Design review of the part built by this model. Coordinates are the model's own, in mm. A direction names the side the tool comes from. Coordinates: 2 decimals unless noted, no trailing zeros. Order: outer loops, then holes, each group sorted by start corner. A loop starts at its lowest first (then second) coordinate and runs counter-clockwise, first axis right, second up. Notation, with made-up numbers: M 38,-27 L 85,-27 A17 ccw 85,0 Z; hole C 70,-38.5 d3. An arc over 180 degrees is marked long. Answer in a Markdown table with one row per item.
from build123d import *

# Parameters (mm, degrees)
SKETCH1_R           = 8.5
SKETCH1_R_2         = 1.5
BOSS_EXTRUDE1_DEPTH = 3
FILLET1_R           = 3


with BuildPart() as part:
    # Sketch1 → Boss-Extrude1 (new body)
    with BuildSketch(Plane(origin=(0, 0, 0), x_dir=(1, 0, 0), z_dir=(0, 1, 0))):
        Polygon((-11, 0), (11, 0), (20.489621783, 17.605313925), (20.489621783, 47.605313925), (8, 62), (-8, 62), (-20.509243816, 47.910305032), (-20.509243816, 17.610706132), align=None)
        with Locations(Location((7.519679741, 17.780252273, 0), (0, 0, 270))):
            Circle(SKETCH1_R, mode=Mode.SUBTRACT)
        with Locations(Location((6, 4, 0), (0, 0, 270))):
            Circle(SKETCH1_R_2, mode=Mode.SUBTRACT)
        with Locations(Location((-6, 4, 0), (0, 0, 90))):
            Circle(SKETCH1_R_2, mode=Mode.SUBTRACT)
        with Locations(Location((-5.25, 57.999859765, 0), (0, 0, 270))):
            Circle(SKETCH1_R_2, mode=Mode.SUBTRACT)
        with Locations(Location((5.25, 57.999859765, 0), (0, 0, 270))):
            Circle(SKETCH1_R_2, mode=Mode.SUBTRACT)
        with Locations(Location((-13.5, 37.605313925, 0), (0, 0, 270))):
            Circle(SKETCH1_R_2, mode=Mode.SUBTRACT)
        with Locations(Location((13.5, 37.605313925, 0), (0, 0, 270))):
            Circle(SKETCH1_R_2, mode=Mode.SUBTRACT)
        with BuildLine():
            Line((-8.730303993, 39.105313925), (8.730303993, 39.105313925))
            ThreePointArc((8.730303993, 39.105313925), (10.179901517, 41.34388933), (12.574074074, 42.518832133))
            ThreePointArc((12.574074074, 42.518832133), (0, 51.105313925), (-12.574074074, 42.518832133))
            ThreePointArc((-12.574074074, 42.518832133), (-10.179901517, 41.34388933), (-8.730303993, 39.105313925))
        make_face(mode=Mode.SUBTRACT)
        with BuildLine():
            Line((-8.730303993, 36.105313925), (8.730303993, 36.105313925))
            ThreePointArc((8.730303993, 36.105313925), (9.667400631, 34.394210987), (11.187975781, 33.171969363))
            ThreePointArc((11.187975781, 33.171969363), (11.998189223, 31.105465162), (10.062695821, 30.018841621))
            ThreePointArc((10.062695821, 30.018841621), (-0.366780245, 27.478383479), (-4.980318958, 17.785955551))
            ThreePointArc((-4.980318958, 17.785955551), (-9.241131059, 13.528058523), (-13.5, 17.787899155))
            Line((-13.5, 17.787899155), (-13.5, 32.605313925))
            ThreePointArc((-13.5, 32.605313925), (-10.541960108, 33.574185051), (-8.730303993, 36.105313925))
        make_face(mode=Mode.SUBTRACT)
    extrude(amount=BOSS_EXTRUDE1_DEPTH)

    # Fillet1
    fillet1_edges = [part.edges().sort_by_distance(p)[0] for p in [
        (-20.509243816, 1.5, -17.610706132),
        (-20.509243816, 1.5, -47.910305032),
        (-8, 1.5, -62),
        (8, 1.5, -62),
        (20.489621783, 1.5, -47.605313925),
        (20.489621783, 1.5, -17.605313925),
    ]]
    fillet(fillet1_edges, radius=FILLET1_R)


solid = part.part
(1) Draft analysis for pull direction X (two halves, no side actions). For faces 1 (the cylindrical face through (-10.21, 1.48, -41.37)), 2 (the flat face through (-15.64, 1.48, -8.59)), 3 (the flat face through (0, 3, -38)), 4 (the cylindrical face through (-0.246, 1.479, -27.576)), state which applies: pulls with the +X half, pulls with the -X half, needs draft (parallel to the pull), parting line crosses it, or undercut.
Return value:
| item | result |
|---|---|
| face 1 | undercut |
| face 2 | pulls with the -X half |
| face 3 | needs draft |
| face 4 | undercut |
(2) For line 1 along X through (y, z) = (1.4, -20); line 2 along Z through (x, y) = (1, 0.55); line 3 along Z through (x, y) = (-6, 2.25), list the stretches that pass through material, from the lowest coordinate up. Write a range as from..to.
Return value:
| item | result |
|---|---|
| line 1 | x = -20.51..-13.5, -4.78..-0.69, 15.72..20.49 |
| line 2 | z = -62..-51.07, -39.11..-36.11, -28.45..-23.23, -12.33..0 |
| line 3 | z = -62..-59.3, -56.7..-49.7, -39.11..-36.11, -15.02..-5.5, -2.5..0 |
(3) Add section D-D, the plane z = -40.5. Give the boundary of the cut face in (x, y), and give its area (3 significant figures).
Return value:
| item | result |
|---|---|
| outline | M -20.51,0 L -9.42,0 L -9.42,3 L -20.51,3 Z; M 9.42,0 L 20.49,0 L 20.49,3 L 9.42,3 Z |
| area | 66.5 mm2 |
(4) Add section C-C, the plane x = 13.5. Give the boundary of the cut face in (y, z).
Return value:
| item | result |
|---|---|
| outline | M 0,-55.66 L 3,-55.66 L 3,-39.11 L 0,-39.11 Z; M 0,-36.11 L 3,-36.11 L 3,-23.82 L 0,-23.82 Z; M 0,-11.74 L 3,-11.74 L 3,-4.64 L 0,-4.64 Z |
(5) Add section A-A, the plane z = -4. Give the boundary of the cut face in (x, y), and give its area (3 significant figures).
Return value:
| item | result |
|---|---|
| outline | M -13.16,0 L -7.5,0 L -7.5,3 L -13.16,3 Z; M -4.5,0 L 4.5,0 L 4.5,3 L -4.5,3 Z; M 7.5,0 L 13.16,0 L 13.16,3 L 7.5,3 Z |
| area | 60.9 mm2 |
(6) Add section B-B, the plane x = -6. Give the boundary of the cut face in (y, z).
Return value:
| item | result |
|---|---|
| outline | M 0,-62 L 3,-62 L 3,-59.3 L 0,-59.3 Z; M 0,-56.7 L 3,-56.7 L 3,-49.7 L 0,-49.7 Z; M 0,-39.11 L 3,-39.11 L 3,-36.11 L 0,-36.11 Z; M 0,-15.02 L 3,-15.02 L 3,-5.5 L 0,-5.5 Z; M 0,-2.5 L 3,-2.5 L 3,0 L 0,0 Z |
(7) For faces 5 (the flat face through (0, 1, -39.105)), 6 (the cylindrical face through (20.305, 1.521, -47.52)), list the 3-axis set-ups (+Z, -Z, +X, -X, +Y, -Y) from which the entire face can be reached by the end or side of a thin tool; tool diameter is ignored.
Return value:
| item | result |
|---|---|
| face 5 | +Y, -Y |
| face 6 | -Z, +X, +Y, -Y |
(8) Insertion check: pin 1 Ø1.5 at (y, z) = (0.5, -17.5) entering from +X; pin 2 Ø1 at (x, y) = (11, 1) entering from -Z. Each pin has a flat end and moves straight along its axis. Give the tip position at first contact, or say it passes through.
Return value:
| item | result |
|---|---|
| pin 1 | stops at x = 20.49 |
| pin 2 | stops at z = -59.12 |
